For this review, use the dimensioned drawing (mm, ordinates from the lowest corner) and the shaded views. A direction names the side the tool comes from. Coordinates: 2 decimals unless noted, no trailing zeros. Loops run counter-clockwise (first coordinate to the right, second up) from the corner with the lowest first, then second, coordinate; pieces in that order, holes last. Notation, with made-up numbers: (57.25, 85) - (111.25, 85) arc R24 ccw to (111.25, 103) - close; hole circle Ø9 at (72.5, -23.75). An arc over 180 degrees is marked (long way). Use a Markdown table: item, result. Add a question column.
1) Add section D-D, the plane y = 34.5. Give the boundary of the cut face in (x, z).
2) Add section B-B, the plane z = 6. Give the boundary of the cut face in (x, y), and give its area (3 significant figures).
3) Add section C-C, the plane x = 14. Give the boundary of the cut face in (y, z), and give its area (4 significant figures).
4) Clearance check with flat-ended pins moving along their axes: pin 1 (15 mm diameter, centred on y = 42.5, z = 31, fed in from +X); pin 2 (5 mm diameter, centred on x = 25.5, z = 37, fed in from -Y); pin 3 (24 mm diameter, centred on y = 13, z = 39.5, fed in from +X). State where each tip first meets the part, or that it passes through.
5) To check wall thickness, follow L1, parallel to X at y = 41, z = 23; L2, parallel to Z at x = 50.5, y = 34; L3, parallel to X at y = 32, z = 45.5. State the ranges of each line that lie inside material, in increasing order. Write a range as [from, to].
6) Add section A-A, the plane y = 43. Give the boundary of the cut face in (x, z), and give its area (3 significant figures).
7) For the marked faces 1, 2 and 3, list the 3-axis set-ups (+Z, -Z, +X, -X, +Y, -Y) from which the entire face can be reached by the end or side of a thin tool; tool diameter is ignored.
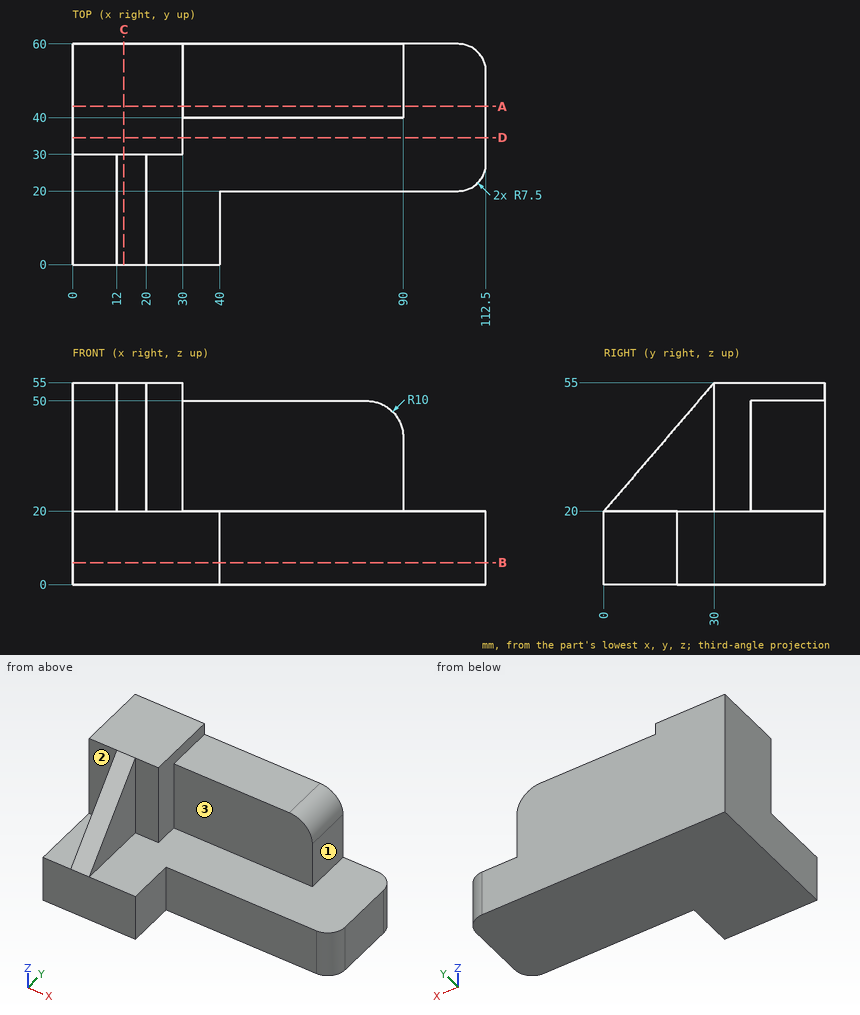
From the geometry:
| question | item | result |
|---|---|---|
| 1 | outline | (0, 0) - (112.5, 0) - (112.5, 20) - (30, 20) - (30, 55) - (0, 55) - close |
| 2 | outline | (0, 0) - (40, 0) - (40, 20) - (105, 20) arc R7.5 ccw to (112.5, 27.5) - (112.5, 52.5) arc R7.5 ccw to (105, 60) - (0, 60) - close |
| 2 | area | 5,280 mm^2 |
| 3 | outline | (0, 0) - (60, 0) - (60, 55) - (30, 55) - (0, 20) - close |
| 3 | area | 2,775 mm^2 |
| 4 | pin 1 | stops at x = 90 |
| 4 | pin 2 | stops at y = 30 |
| 4 | pin 3 | stops at x = 20 |
| 5 | L1 | x = [0, 90] |
| 5 | L2 | z = [0, 20] |
| 5 | L3 | x = [0, 30] |
| 6 | outline | (0, 0) - (112.5, 0) - (112.5, 20) - (90, 20) - (90, 40) arc R10 ccw to (80, 50) - (30, 50) - (30, 55) - (0, 55) - close |
| 6 | area | 5,080 mm^2 |
| 7 | face 1 | +Z, +X, +Y, -Y |
| 7 | face 2 | +Z, -X, -Y |
| 7 | face 3 | +Z, +X, -Y |
